The figure shows three views and two pictorial views of one solid part (mm, origin at its lowest corner). Answer the questions. Give positions to 0.01 mm unless a question says otherwise; leave off trailing zeros. Order: outer loops, then holes, each group sorted by start corner. A loop starts at its lowest first (then second) coordinate and runs counter-clockwise, first axis right, second up. Notation, with made-up numbers: M 0.5,40.25 L 31.5,40.25 A18 ccw 31.5,50.25 Z; hole C -30,19 d6. An arc over 180 degrees is marked long. Write item = value, one per line. Start each with the question number.
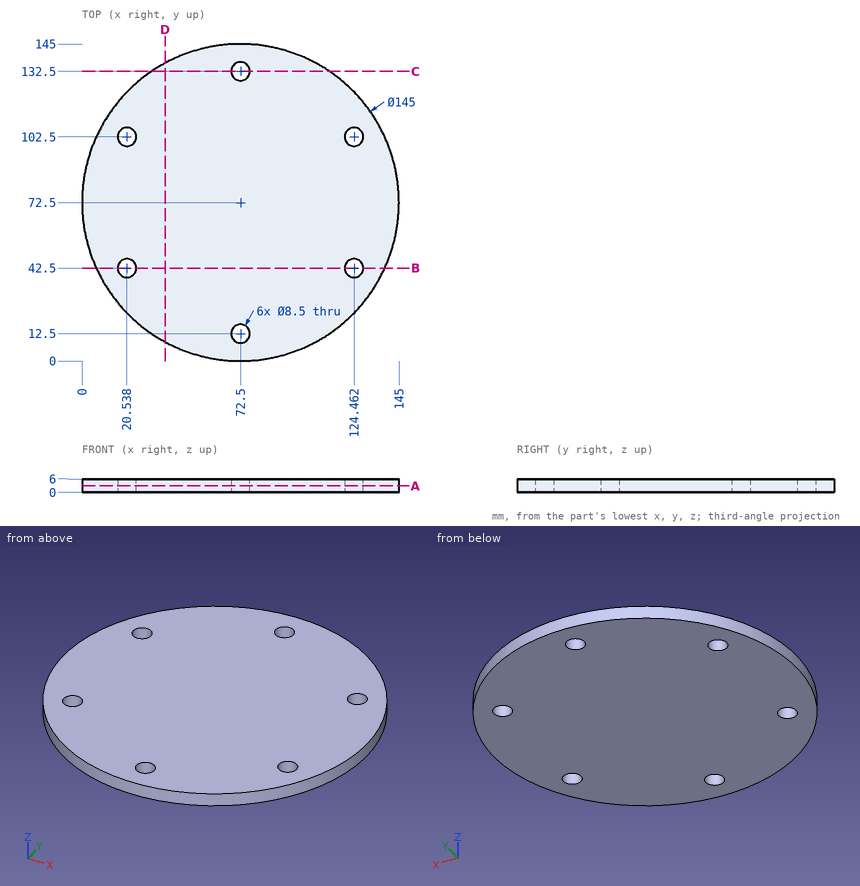
1) Find section B-B on y = 42.5. Determine the outline of the cut face in (x, z).
2) Find section A-A on z = 2.85. Determine the outline of the cut face in (x, y).
3) Each of these flat-tipped pins is pushed along its axis until it touches: P1, Ø3, axis at x = 34, z = 1.5, coming from the -Y side; P2, Ø2, axis at y = 26, z = 3, coming from the -X side (1 decimal); P3, Ø1.5, axis at y = 70.5, z = 1, coming from the -X side. Where does it stop, or does it pass through?
4) Find section C-C on y = 132.5. Determine the outline of the cut face in (x, z).
5) Find the intervals of material crossed by probe 1 along Y at (x, z) = (72.5, 3.6); probe 2 along X at (y, z) = (105, 1.1) (1 decimal); probe 3 along X at (y, z) = (71.5, 3.8), in increasing order. Write a range as [from, to].
6) Find section D-D on x = 38. Determine the outline of the cut face in (y, z) (1 decimal), plus the area to 3 significant figures.
Numbers:
q1.outline = M 6.5,0 L 16.29,0 L 16.29,6 L 6.5,6 Z; M 24.79,0 L 120.21,0 L 120.21,6 L 24.79,6 Z; M 128.71,0 L 138.5,0 L 138.5,6 L 128.71,6 Z
q2.outline = C 72.5,72.5 d145; hole C 20.54,42.5 d8.5; hole C 20.54,102.5 d8.5; hole C 72.5,12.5 d8.5; hole C 72.5,132.5 d8.5; hole C 124.46,42.5 d8.5; hole C 124.46,102.5 d8.5
q3.P1 = 10.15
q3.P2 = 16.1
q3.P3 = 0.01
q4.outline = M 31.8,0 L 68.25,0 L 68.25,6 L 31.8,6 Z; M 76.75,0 L 113.2,0 L 113.2,6 L 76.75,6 Z
q5.probe_1 = [0, 8.25], [16.75, 128.25], [136.75, 145]
q5.probe_2 = [7.7, 17.1], [24, 121], [127.9, 137.3]
q5.probe_3 = [0.01, 144.99]
q6.outline = M 8.7,0 L 136.3,0 L 136.3,6 L 8.7,6 Z
q6.area = 765 mm2
